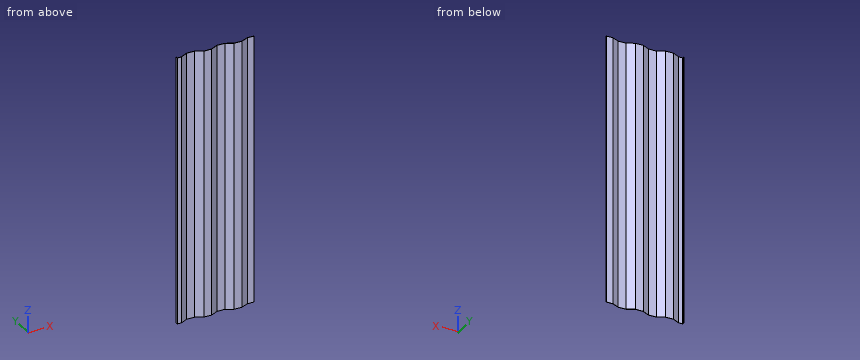
from build123d import *

# Parameters (mm, degrees)
EXTRUDE_THIN1_DEPTH = 2530


with BuildPart() as part:
    # Sketch1 → Extrude-Thin1 (new body)
    with BuildSketch(Plane.XY):
        Polygon((0, 20), (0, 0), (40, 0), (107.973084028, 35.696369631), (182.973084028, 35.696369631), (250.946168056, 0), (325.946168056, 0), (393.919252083, 35.696369631), (468.919252083, 35.696369631), (536.892336111, 0), (611.892336111, 0), (679.865420139, 31.696369631), (742.000000002, 31.696369631), (742.000000002, 33.696369631), (679.422030814, 33.696369631), (611.448946786, 2), (537.385552948, 2), (469.41246892, 37.696369631), (393.426035246, 37.696369631), (325.452951219, 2), (251.439384892, 2), (183.466300865, 37.696369631), (107.479867191, 37.696369631), (39.506783163, 2), (2, 2), (2, 20), align=None)
    extrude(amount=EXTRUDE_THIN1_DEPTH)


solid = part.part
Can you work these out from the model? Positions are in its coordinate system, mm. Coordinates: 2 decimals unless noted, no trailing zeros. Loops run counter-clockwise (first coordinate to the right, second up) from the corner with the lowest first, then second, coordinate; pieces in that order, holes last. Notation, with made-up numbers: (59, 14) - (111, 14) arc R9 cw to (111, 23) - close; hole circle Ø6 at (45.5, 24.25). An arc over 180 degrees is marked (long way). Put each result on its own line as item: value. Start each with the question number.
Item 1: For pin 1 (4 mm diameter, centred on y = 29, z = 1373, fed in from -X); pin 2 (20 mm diameter, centred on y = 10, z = 637, fed in from +X); pin 3 (1 mm diameter, centred on x = 81, z = 1045, fed in from -Y), each with a flat end and sliding along its axis, tell me the tip position at first contact or that it passes through.
Item 2: If I drill on line 1 along X through (y, z) = (25.5, 978.5); line 2 along X through (y, z) = (6.5, 1577.5); line 3 along X through (y, z) = (10, 651) (3 decimals), over which ranges is the centre line in solid material (lowest first)?
Item 3: Suppose I cut it at A-A (z = 1677.5). Please give me the cut outline in (x, y), and give its area (3 significant figures).
Here are the results:
1. pin 1: x = 87.11
1. pin 2: x = 654.78
1. pin 3: y = 21.27
2. line 1: 84.26 to 88.56, 202.39 to 206.69, 370.2 to 374.5, 488.34 to 492.64, 661.84 to 666.58
2. line 2: 0 to 2, 48.08 to 52.38, 238.57 to 242.87, 334.02 to 338.32, 524.52 to 528.82, 621.1 to 625.83
2. line 3: 0 to 2, 54.74 to 59.042, 231.904 to 236.206, 340.687 to 344.988, 517.85 to 522.152, 628.605 to 633.337
3. outline: (0, 0) - (40, 0) - (107.97, 35.7) - (182.97, 35.7) - (250.95, 0) - (325.95, 0) - (393.92, 35.7) - (468.92, 35.7) - (536.89, 0) - (611.89, 0) - (679.87, 31.7) - (742, 31.7) - (742, 33.7) - (679.42, 33.7) - (611.45, 2) - (537.39, 2) - (469.41, 37.7) - (393.43, 37.7) - (325.45, 2) - (251.44, 2) - (183.47, 37.7) - (107.48, 37.7) - (39.51, 2) - (2, 2) - (2, 20) - (0, 20) - close
3. area: 1,600 mm²
